Read the model definition and answer for the solid it produces. Units are mm, in the model's axes. Coordinates: 2 decimals unless noted, no trailing zeros. Loops run counter-clockwise (first coordinate to the right, second up) from the corner with the lowest first, then second, coordinate; pieces in that order, holes last. Notation, with made-up numbers: (70, 82.25) -> (109, 82.25) arc R37 ccw to (109, 120.25) -> close; hole circle Ø11 at (59.25, 77). An arc over 180 degrees is marked (long way). Answer as a JSON object with one key per item and string values. Group by question number.
Q1. This flat-tipped pin is pushed along its axis until it touches: P1, Ø10.5, axis at x = -110, y = -30, coming from the -Z side. Where does it stop, or does it pass through?
Q2. The part is cut by section C-C on x = 0. Write down the section's boundary in (y, z), and give its area (3 significant figures).
Q3. Straight lines are drawn through the part: line 1 along Y through (x, z) = (0, 0.5); line 2 along X through (y, z) = (-29.5, 0.5); line 3 along Y through (x, z) = (72.5, 4). For each, find the intervals that lie inside material, in ascending order. Write a range as [from, to].
Q4. The part is cut by section B-B on y = -30. Write down the section's boundary in (x, z), and give its area (3 significant figures).
Q5. The part is cut by section A-A on x = -110. Write down the section's boundary in (y, z), and give its area (3 significant figures).
Q6. The part is cut by section D-D on z = -0.5. State how many separate pieces and enclosed holes the cut face has, and give its area (3 significant figures).
from build123d import *

# Parameters (mm, degrees)
SKETCH_1_W              = 250
SKETCH_1_H              = 170
EXTRUDE_1_DEPTH         = 5
SKETCH_2_W              = 80
SKETCH_2_H              = 40
CUT_EXTRUDE_1_DEPTH     = 10
HOLE_WIZARD_9_0_9_1_D   = 9
PATTERN_LINEAR_1_COUNT  = 3
PATTERN_LINEAR_1_PITCH  = 110
HOLE_WIZARD_12_0_12_1_D = 12
SKETCH_7_R              = 17.5
CUT_EXTRUDE_2_DEPTH     = 10
HOLE_WIZARD_M8_1_D      = 6.8
FILLET_1_R              = 10


with BuildPart() as part:
    # 草图1 → 凸台-拉伸1 (new, symmetric)
    with BuildSketch(Plane.XY):
        Rectangle(SKETCH_1_W, SKETCH_1_H)
    extrude(amount=EXTRUDE_1_DEPTH, both=True)

    # 草图2 → 切除-拉伸1 (cut)
    with BuildSketch(Plane.XY.offset(5)):
        with Locations((85, 65)):
            Rectangle(SKETCH_2_W, SKETCH_2_H)
    cut_extrude_1 = extrude(amount=-CUT_EXTRUDE_1_DEPTH, mode=Mode.SUBTRACT)

    # 镜向1: 切除-拉伸1 across plane
    add(cut_extrude_1.mirror(Plane(origin=(0, 0, 0), x_dir=(0, 0, 1), z_dir=(1, 0, 0))), mode=Mode.SUBTRACT)

    # Ø9.0 (9) 直径孔1 (through all)
    with Locations(Plane.XY.offset(5)):
        with Locations((-110, -30), (-110, -70)):
            hole_wizard_9_0_9_1 = Hole(HOLE_WIZARD_9_0_9_1_D / 2)

    # 阵列(线性)1: Ø9.0 (9) 直径孔1 ×3
    with Locations(*[(i * PATTERN_LINEAR_1_PITCH, 0, 0) for i in range(1, PATTERN_LINEAR_1_COUNT)]):
        add(hole_wizard_9_0_9_1, mode=Mode.SUBTRACT)

    # Ø12.0 (12) 直径孔1 (through all)
    with Locations(Plane.XY.offset(5)):
        with Locations((-100, 35), (100, 35)):
            Hole(HOLE_WIZARD_12_0_12_1_D / 2)

    # 草图7 → 切除-拉伸2 (cut)
    with BuildSketch(Plane.XY.offset(5)):
        with Locations((0, 35)):
            Circle(SKETCH_7_R)
    extrude(amount=-CUT_EXTRUDE_2_DEPTH, mode=Mode.SUBTRACT)

    # M8 螺纹孔1 (through all)
    with Locations(Plane.XY.offset(5)):
        with Locations((-26.515, 8.485), (26.515, 61.515)):
            Hole(HOLE_WIZARD_M8_1_D / 2)

    # 圆角1
    fillet_1_edges = [part.edges().sort_by_distance(p)[0] for p in [
        (45, 85, 0),
        (125, 45, 0),
        (-45, 85, 0),
        (-125, 45, 0),
        (125, -85, 0),
        (-125, -85, 0),
    ]]
    fillet(fillet_1_edges, radius=FILLET_1_R)


solid = part.part
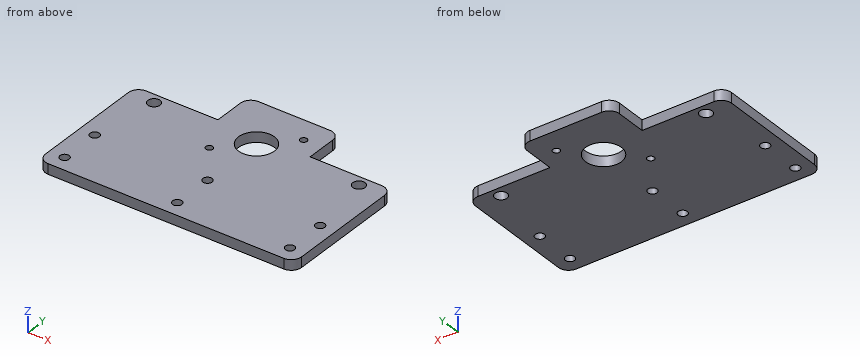
Final values:
{
 "1": {"P1": "stops at z = -5"},
 "2": {"outline": "(-85, -5) -> (-74.5, -5) -> (-74.5, 5) -> (-85, 5) -> close; (-65.5, -5) -> (-34.5, -5) -> (-34.5, 5) -> (-65.5, 5) -> close; (-25.5, -5) -> (17.5, -5) -> (17.5, 5) -> (-25.5, 5) -> close; (52.5, -5) -> (85, -5) -> (85, 5) -> (52.5, 5) -> close", "area": "1,170 mm2"},
 "3": {"line 1": "y = [-85, -74.5], [-65.5, -34.5], [-25.5, 17.5], [52.5, 85]", "line 2": "x = [-125, -114.47], [-105.53, -4.47], [4.47, 105.53], [114.47, 125]", "line 3": "y = [-85, 45]"},
 "4": {"outline": "(-125, -5) -> (-114.5, -5) -> (-114.5, 5) -> (-125, 5) -> close; (-105.5, -5) -> (-4.5, -5) -> (-4.5, 5) -> (-105.5, 5) -> close; (4.5, -5) -> (105.5, -5) -> (105.5, 5) -> (4.5, 5) -> close; (114.5, -5) -> (125, -5) -> (125, 5) -> (114.5, 5) -> close", "area": "2,230 mm2"},
 "5": {"outline": "(-85, -5) -> (-74.5, -5) -> (-74.5, 5) -> (-85, 5) -> close; (-65.5, -5) -> (-34.5, -5) -> (-34.5, 5) -> (-65.5, 5) -> close; (-25.5, -5) -> (45, -5) -> (45, 5) -> (-25.5, 5) -> close", "area": "1,120 mm2"},
 "6": {"separate pieces": "1", "enclosed holes": "11", "area": "34,300 mm2"}
}
